Geometry: final body of the model. Coordinates: model frame, mm. A direction names the side the tool comes from. Give positions to 0.01 mm unless a question says otherwise; leave off trailing zeros. Loops run counter-clockwise (first coordinate to the right, second up) from the corner with the lowest first, then second, coordinate; pieces in that order, holes last.
from build123d import *

# Parameters (mm, degrees)
EXTRUDE_1_DEPTH = 7
SKETCH_2_W      = 30
SKETCH_2_H      = 65
EXTRUDE_2_DEPTH = 4
FILLET_1_R      = 3
SKETCH_3_W      = 15
SKETCH_3_H      = 30
EXTRUDE_3_DEPTH = 4


with BuildPart() as part:
    # 草图1 → 凸台-拉伸1 (new body)
    with BuildSketch(Plane.XY):
        Polygon((0, 0), (-15, 0), (-15, 25), (15, 25), (15, 0), align=None)
        with BuildLine():
            Line((-8, 15.5), (8, 15.5))
            ThreePointArc((8, 15.5), (11, 12.5), (8, 9.5))
            Line((8, 9.5), (-8, 9.5))
            ThreePointArc((-8, 9.5), (-11, 12.5), (-8, 15.5))
        make_face(mode=Mode.SUBTRACT)
    extrude(amount=EXTRUDE_1_DEPTH)

    # 草图2 → 凸台-拉伸2 (add)
    with BuildSketch(Plane.XY.offset(7)):
        with Locations((0, 32.5)):
            Rectangle(SKETCH_2_W, SKETCH_2_H)
        with BuildLine():
            Line((-8, 9.5), (8, 9.5))
            ThreePointArc((8, 9.5), (11, 12.5), (8, 15.5))
            Line((8, 15.5), (-8, 15.5))
            ThreePointArc((-8, 15.5), (-11, 12.5), (-8, 9.5))
        make_face(mode=Mode.SUBTRACT)
    extrude(amount=EXTRUDE_2_DEPTH)

    # 圆角1
    fillet_1_edges = [part.edges().sort_by_distance(p)[0] for p in [
        (-15, 65, 9),
        (15, 65, 9),
    ]]
    fillet(fillet_1_edges, radius=FILLET_1_R)

    # 草图3 → 凸台-拉伸3 (add)
    with BuildSketch(Plane.XY.offset(11)):
        with Locations((0, 80)):
            Rectangle(SKETCH_3_W, SKETCH_3_H)
    extrude(amount=-EXTRUDE_3_DEPTH)


solid = part.part
Item 1: Section query D-D on z = 8.5. Return loops of the section in (x, y).
Values follow:
outline: (-15, 0) - (15, 0) - (15, 62) arc R3 ccw to (12, 65) - (7.5, 65) - (7.5, 95) - (-7.5, 95) - (-7.5, 65) - (-12, 65) arc R3 ccw to (-15, 62) - close; hole (-8, 9.5) - (8, 9.5) arc R3 ccw to (8, 15.5) - (-8, 15.5) arc R3 ccw to start
Item 2: Pin query (flat end, axial travel): pin 1 (3 mm diameter, centred on y = 82.5, z = 9, fed in from -X); pin 2 (4 mm diameter, centred on x = 2, z = 8.5, fed in from -Y); pin 3 (1.2 mm diameter, centred on x = -9, z = 9.5, fed in from +Y); pin 4 (1.2 mm diameter, centred on y = 87, z = 10, fed in from +X). Return the tip coordinate at first contact, or that it passes through.
Values follow:
pin 1: stops at x = -7.5
pin 2: stops at y = 0
pin 3: stops at y = 65
pin 4: stops at x = 7.5
Item 3: Ray query, probe 1 along Y at (x, z) = (4, 4.5); probe 2 along Y at (x, z) = (2.75, 7.5); probe 3 along Z at (x, y) = (1.5, 85). Return the intervals inside material, ascending.
Values follow:
probe 1: y = 0 to 9.5, 15.5 to 25
probe 2: y = 0 to 9.5, 15.5 to 95
probe 3: z = 7 to 11
Item 4: Section query A-A on x = -2.25. Return loops of the section in (y, z).
Values follow:
outline: (0, 0) - (9.5, 0) - (9.5, 11) - (0, 11) - close; (15.5, 0) - (25, 0) - (25, 7) - (95, 7) - (95, 11) - (15.5, 11) - close
Item 5: Section query B-B on y = 12.5. Return loops of the section in (x, z).
Values follow:
outline: (-15, 0) - (-11, 0) - (-11, 11) - (-15, 11) - close; (11, 0) - (15, 0) - (15, 11) - (11, 11) - close
Item 6: Set-up query: faces 5 (the face through (0, 25, 3)), 6 (the face through (-10, 65, 9)), 7 (the face through (10, 65, 9)), 8 (the face through (11, 12.4, 5.4)), 9 (the face through (15, 24, 7)). Return all of +Z, -Z, +X, -X, +Y, -Y with unobstructed straight access to the full face (end or side cutting, diameter ignored); none if empty.
Values follow:
face 5: -Z, +X, -X, +Y
face 6: +Z, -Z, -X, +Y
face 7: +Z, -Z, +X, +Y
face 8: +Z, -Z
face 9: +Z, -Z, +X, +Y, -Y
Item 7: Section query C-C on z = 3.25. Return loops of the section in (x, y).
Values follow:
outline: (-15, 0) - (15, 0) - (15, 25) - (-15, 25) - close; hole (-8, 9.5) - (8, 9.5) arc R3 ccw to (8, 15.5) - (-8, 15.5) arc R3 ccw to start
Item 8: Draft query along X for faces 1 (the face through (0, 15.5, 5)), 2 (the face through (-7.5, 80, 9)), 3 (the face through (0, 0, 5)), 4 (the face through (7.5, 80, 9)). Return one class per face: +X half, -X half, draft (parallel to the pull), parting line (faces both ways), or undercut.
Values follow:
face 1: undercut
face 2: -X half
face 3: draft
face 4: +X half
